The model under review builds one solid part; all positions refer to its coordinate system, in mm. Face numbers are marked on the shaded views. A direction names the side the tool comes from. Round coordinates to 2 decimals unless told otherwise and drop trailing zeros. Order: outer loops, then holes, each group sorted by start corner. A loop starts at its lowest first (then second) coordinate and runs counter-clockwise, first axis right, second up. Notation, with made-up numbers: M 76.5,-2.75 L 133.5,-2.75 A9 ccw 133.5,7.25 Z; hole C -16,50 d2. An arc over 180 degrees is marked long. Answer as a JSON object with one key per item and string values. Group by question number.
1. Add section B-B on x = -22.5. State the section outline as (y, z) points, and give its area (3 significant figures).
2. Mouldability with a two-part tool opening along Y and no side actions: class the marked faces 1, 2 and 3 as released by +Y, released by -Y, zero draft, split by the parting line, or undercut.
3. Machinability: for the marked faces 4 and 5, which of the approach directions +Z, -Z, +X, -X, +Y, -Y give a long, thin tool a straight path to every point of the face, cutting with its end or side? Answer none if there is none.
4. Add section C-C on y = 7.5. State the section outline as (x, z) points.
5. Add section A-A on z = 1. State the section outline as (x, y) points, and give its area (3 significant figures).
6. Clearance check with flat-ended pins moving along their axes: P1, Ø6.5, axis at x = -22.5, y = -9, coming from the +Z side; P2, Ø2.5, axis at x = 21.5, y = -8.5, coming from the +Z side. State where each tip first meets the part, or that it passes through.
7. To check wall thickness, follow probe 1 along Y at (x, z) = (22.5, 6.35); probe 2 along Y at (x, z) = (-22.5, 1); probe 3 along X at (y, z) = (-6.25, 4.25). State the ranges of each line that lie inside material, in increasing order. Write a range as [from, to].
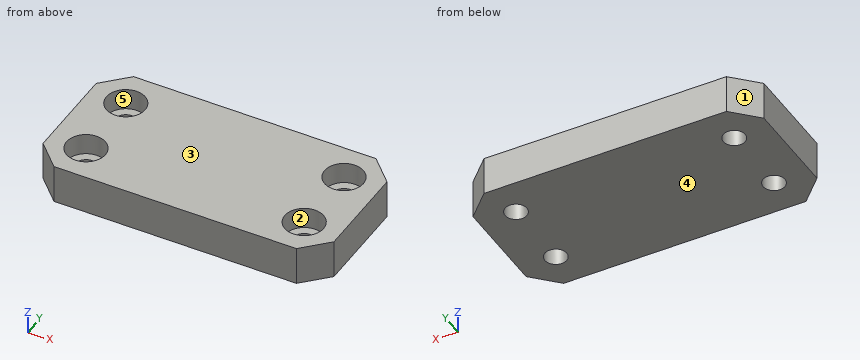
```python
from build123d import *

# Parameters (mm, degrees)
SKETCH1_W                                           = 60
SKETCH1_H                                           = 30
BOSS_EXTRUDE1_DEPTH                                 = 8
CBORE_FOR_M4_HEX_SOCKET_HEAD_CAP_SCREW1_D           = 4.5
CBORE_FOR_M4_HEX_SOCKET_HEAD_CAP_SCREW1_CBORE_D     = 8
CBORE_FOR_M4_HEX_SOCKET_HEAD_CAP_SCREW1_CBORE_DEPTH = 4.4
CHAMFER1_SIZE                                       = 5


with BuildPart() as part:
    # Sketch1 → Boss-Extrude1 (new body)
    with BuildSketch(Plane.XY):
        Rectangle(SKETCH1_W, SKETCH1_H)
    extrude(amount=BOSS_EXTRUDE1_DEPTH)

    # CBORE for M4 Hex Socket Head Cap Screw1 (through all)
    with Locations(Plane.XY.offset(8)):
        with Locations((22.5, 7.5), (-22.5, 7.5), (-22.5, -7.5), (22.5, -7.5)):
            CounterBoreHole(CBORE_FOR_M4_HEX_SOCKET_HEAD_CAP_SCREW1_D / 2, CBORE_FOR_M4_HEX_SOCKET_HEAD_CAP_SCREW1_CBORE_D / 2, CBORE_FOR_M4_HEX_SOCKET_HEAD_CAP_SCREW1_CBORE_DEPTH)

    # Chamfer1
    chamfer1_edges = [part.edges().sort_by_distance(p)[0] for p in [
        (30, -15, 4),
        (-30, -15, 4),
        (-30, 15, 4),
        (30, 15, 4),
    ]]
    chamfer(chamfer1_edges, length=CHAMFER1_SIZE)


solid = part.part
```
Recorded:
{
 "1": {"outline": "M -15,0 L -9.75,0 L -9.75,3.6 L -11.5,3.6 L -11.5,8 L -15,8 Z; M -5.25,0 L 5.25,0 L 5.25,3.6 L 3.5,3.6 L 3.5,8 L -3.5,8 L -3.5,3.6 L -5.25,3.6 Z; M 9.75,0 L 15,0 L 15,8 L 11.5,8 L 11.5,3.6 L 9.75,3.6 Z", "area": "137 mm²"},
 "2": {"face 1": "released by +Y", "face 2": "undercut", "face 3": "zero draft"},
 "3": {"face 4": "-Z, +X, -X, +Y, -Y", "face 5": "+Z"},
 "4": {"outline": "M -30,0 L -24.75,0 L -24.75,3.6 L -26.5,3.6 L -26.5,8 L -30,8 Z; M -20.25,0 L 20.25,0 L 20.25,3.6 L 18.5,3.6 L 18.5,8 L -18.5,8 L -18.5,3.6 L -20.25,3.6 Z; M 24.75,0 L 30,0 L 30,8 L 26.5,8 L 26.5,3.6 L 24.75,3.6 Z"},
 "5": {"outline": "M -30,-10 L -25,-15 L 25,-15 L 30,-10 L 30,10 L 25,15 L -25,15 L -30,10 Z; hole C -22.5,-7.5 d4.5; hole C -22.5,7.5 d4.5; hole C 22.5,-7.5 d4.5; hole C 22.5,7.5 d4.5", "area": "1,690 mm²"},
 "6": {"P1": "stops at z = 8", "P2": "stops at z = 3.6"},
 "7": {"probe 1": "y = [-15, -11.5], [-3.5, 3.5], [11.5, 15]", "probe 2": "y = [-15, -9.75], [-5.25, 5.25], [9.75, 15]", "probe 3": "x = [-30, -26.3], [-18.7, 18.7], [26.3, 30]"}
}
